Source: CAD feature listing. Evaluate the final solid. Frame: model axes, mm. Coordinates: 2 decimals unless noted, no trailing zeros. Loops run counter-clockwise (first coordinate to the right, second up) from the corner with the lowest first, then second, coordinate; pieces in that order, holes last.
from build123d import *

# Parameters (mm, degrees)
SKETCH_1_W          = 80
SKETCH_1_H          = 180
EXTRUDE_1_DEPTH     = 5
CHAMFER_1_SIZE      = 5
SKETCH_2_R          = 3.5
CUT_EXTRUDE_1_DEPTH = 5


with BuildPart() as part:
    # 草图1 → 凸台-拉伸1 (new body)
    with BuildSketch(Plane.XY):
        Rectangle(SKETCH_1_W, SKETCH_1_H)
    extrude(amount=EXTRUDE_1_DEPTH)

    # 倒角1
    chamfer_1_edges = [part.edges().sort_by_distance(p)[0] for p in [
        (40, -90, 2.5),
        (-40, -90, 2.5),
        (-40, 90, 2.5),
        (40, 90, 2.5),
    ]]
    chamfer(chamfer_1_edges, length=CHAMFER_1_SIZE)

    # 草图2 → 切除-拉伸1 (cut)
    with BuildSketch(Plane.XY.offset(5)):
        with Locations((-30, 75)):
            Circle(SKETCH_2_R)
        with Locations((30, 75)):
            Circle(SKETCH_2_R)
        with Locations((-30, -75)):
            Circle(SKETCH_2_R)
        with Locations((30, -75)):
            Circle(SKETCH_2_R)
    extrude(amount=-CUT_EXTRUDE_1_DEPTH, mode=Mode.SUBTRACT)


solid = part.part
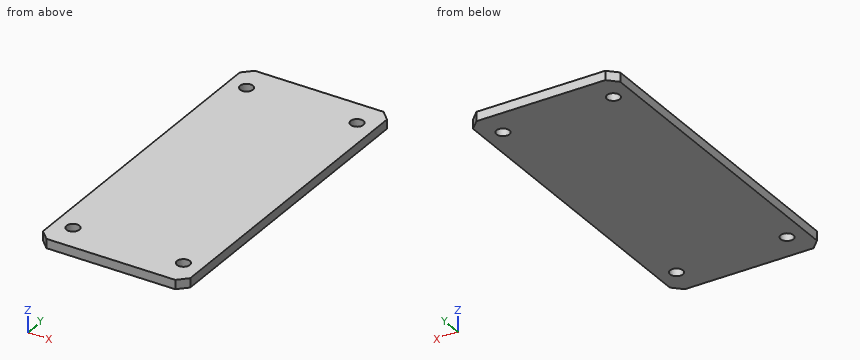
Q1. Section A-A, the plane y = 75. Return the cut outline in (x, z).
Q2. Contact query for a flat-ended pin moving along its axis: pin 1 Ø12 at (x, y) = (-17.5, -4) entering from -Z. Output: stop coordinate, or through.
Q3. Line query: line 1 along Y through (x, z) = (30, 1.65); line 2 along Y through (x, z) = (27.5, 4.3); line 3 along Y through (x, z) = (-36, 1.3). Output: solid intervals per line, ascending.
Q4. Section B-B, the plane x = 30. Return the cut outline in (y, z), plus the area to 3 significant figures.
Derived:
1. outline: (-40, 0) - (-33.5, 0) - (-33.5, 5) - (-40, 5) - close; (-26.5, 0) - (26.5, 0) - (26.5, 5) - (-26.5, 5) - close; (33.5, 0) - (40, 0) - (40, 5) - (33.5, 5) - close
2. pin 1: stops at z = 0
3. line 1: y = -90 to -78.5, -71.5 to 71.5, 78.5 to 90
3. line 2: y = -90 to -77.45, -72.55 to 72.55, 77.45 to 90
3. line 3: y = -89 to 89
4. outline: (-90, 0) - (-78.5, 0) - (-78.5, 5) - (-90, 5) - close; (-71.5, 0) - (71.5, 0) - (71.5, 5) - (-71.5, 5) - close; (78.5, 0) - (90, 0) - (90, 5) - (78.5, 5) - close
4. area: 830 mm2
